Part print with two shaded views. Sizes in mm from the minimum x, y, z corner. A direction names the side the tool comes from. Round coordinates to 2 decimals unless told otherwise and drop trailing zeros. Order: outer loops, then holes, each group sorted by start corner. A loop starts at its lowest first (then second) coordinate and runs counter-clockwise, first axis right, second up. Notation, with made-up numbers: M 10.25,81 L 19.25,81 A22 cw 19.25,100 Z; hole C 41.25,-29 d9. An arc over 180 degrees is marked long. Answer as a JSON object with one key per item and string values.
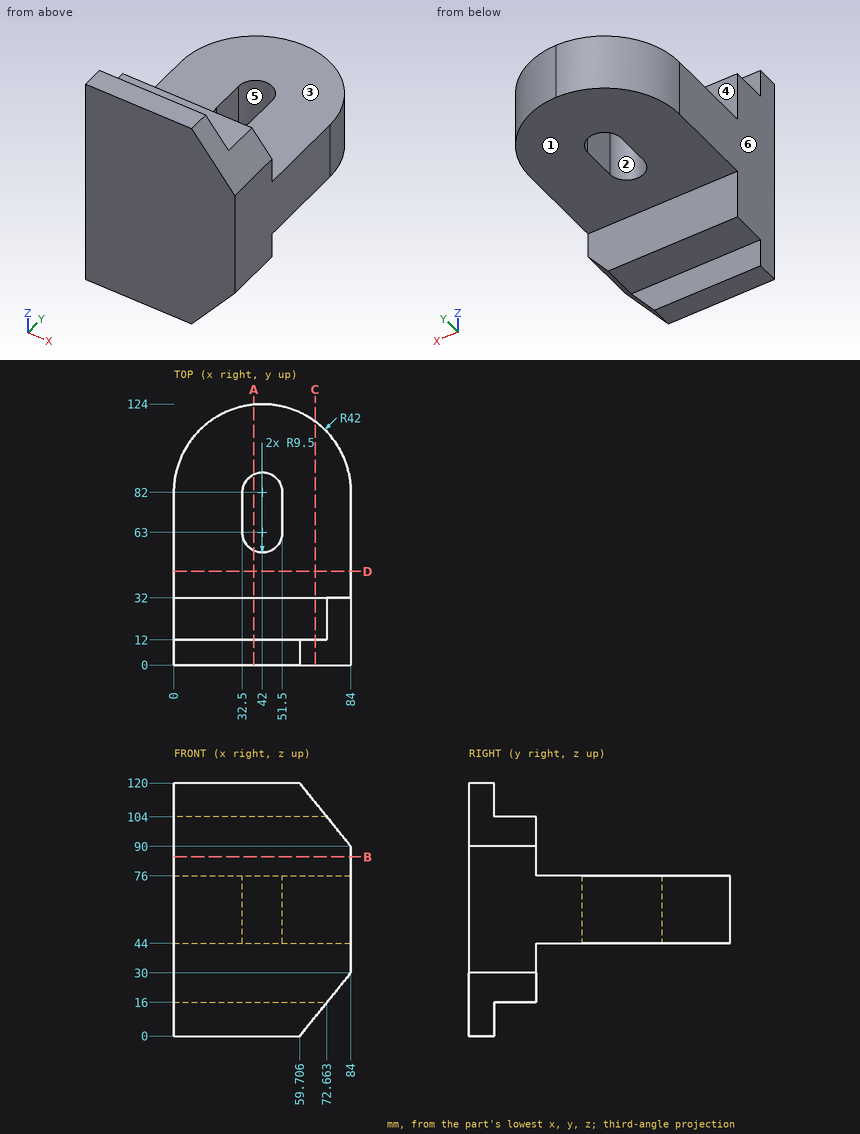
Item 1: Two-plate mould, pull along Y, no slides. Class the marked faces 4, 5 and 6: released by +Y, released by -Y, zero draft, split by the parting line, or undercut.
Worked answers:
{"face 4": "released by +Y", "face 5": "undercut", "face 6": "zero draft"}
Item 2: Saw through at A-A on x = 38. List the corners of the cut face in (y, z), and give its area (3 significant figures).
Worked answers:
{"outline": "M 0,0 L 12,0 L 12,16 L 32,16 L 32,44 L 54.38,44 L 54.38,76 L 32,76 L 32,104 L 12,104 L 12,120 L 0,120 Z; M 90.62,44 L 123.81,44 L 123.81,76 L 90.62,76 Z", "area": "4,980 mm2"}
Item 3: Saw through at C-C on x = 67. List the corners of the cut face in (y, z).
Worked answers:
{"outline": "M 0,9.01 L 12,9.01 L 12,16 L 32,16 L 32,44 L 115.75,44 L 115.75,76 L 32,76 L 32,104 L 12,104 L 12,110.99 L 0,110.99 Z"}
Item 4: Drop flat-ended pins along their axis: pin 1 Ø22.5 at (x, z) = (59.5, 29) entering from +Y; pin 2 Ø10 at (x, y) = (75, 33) entering from -Z; pin 3 Ø10 at (x, y) = (41, 91.5) entering from +Z. Give the stop position or say it passes through.
Worked answers:
{"pin 1": "stops at y = 32", "pin 2": "stops at z = 16", "pin 3": "stops at z = 76"}
Item 5: Wall check: line 1 along X through (y, z) = (80.5, 55); line 2 along Z through (x, y) = (6, 56.5); line 3 along Z through (x, y) = (32, 23.5). Give the ranges that are in metal, low to high. Write a range as [from, to].
Worked answers:
{"line 1": "x = [0, 32.5], [51.5, 84]", "line 2": "z = [44, 76]", "line 3": "z = [16, 104]"}
Item 6: 3-axis set-ups, long thin cutter, end or side, ignore diameter. For the marked faces 1, 2 and 3: which of +Z, -Z, +X, -X, +Y, -Y reach the whole face in a straight line?
Worked answers:
{"face 1": "-Z, +X, -X, +Y", "face 2": "+Z, -Z", "face 3": "+Z, +X, -X, +Y"}
Item 7: Saw through at B-B on z = 85. List the corners of the cut face in (x, y), and give its area (3 significant figures).
Worked answers:
{"outline": "M 0,0 L 84,0 L 84,32 L 0,32 Z", "area": "2,690 mm2"}
Item 8: Saw through at D-D on y = 44.5. List the corners of the cut face in (x, z).
Worked answers:
{"outline": "M 0,44 L 84,44 L 84,76 L 0,76 Z"}
